```python
from build123d import *

# Parameters (mm, degrees)
SKETCH_1_R               = 21
EXTRUDE_1_DEPTH          = 25
CUT_EXTRUDE_1_DEPTH      = 396.281407624
CUT_EXTRUDE_1_DEPTH_BACK = 396.281407624
SKETCH_2_W               = 10
SKETCH_2_H               = 16.9


with BuildPart() as part:
    # 草图1 → 凸台-拉伸1 (new, symmetric)
    with BuildSketch(Plane.XY):
        with BuildLine():
            Line((0, 0), (0, 121.205505282))
            ThreePointArc((0, 121.205505282), (5, 143), (0, 164.794494718))
            Line((0, 164.794494718), (0, 370))
            Line((0, 370), (-15, 385))
            Line((-15, 385), (-90, 374.459437397))
            Line((-90, 374.459437397), (-90, 164.794494718))
            ThreePointArc((-90, 164.794494718), (-95, 143), (-90, 121.205505282))
            Line((-90, 121.205505282), (-90, 90))
            ThreePointArc((-90, 90), (-63.639610307, 26.360389693), (0, 0))
        make_face()
        with Locations((-45, 143)):
            Circle(SKETCH_1_R, mode=Mode.SUBTRACT)
    extrude(amount=EXTRUDE_1_DEPTH, both=True)

    # 草图2 → 切除-拉伸1 (cut, two sides: drawn at the far end of the back side and taken through both)
    with BuildSketch(Plane(origin=(-36.649271725, -5.150719239, 0), x_dir=(0, 0, -1), z_dir=(0.9902680687415697, 0.1391731009600695, 0)).offset(-CUT_EXTRUDE_1_DEPTH_BACK)):
        with Locations((-20, 374.89080298)):
            Rectangle(SKETCH_2_W, SKETCH_2_H)
        with Locations((20, 374.89080298)):
            Rectangle(SKETCH_2_W, SKETCH_2_H)
    extrude(amount=CUT_EXTRUDE_1_DEPTH + CUT_EXTRUDE_1_DEPTH_BACK, mode=Mode.SUBTRACT)


solid = part.part
```
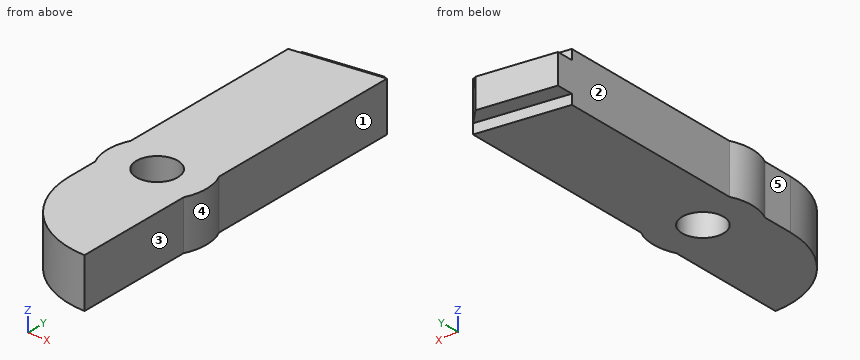
The listing builds one solid part. Answer for the finished solid, in the listing's coordinates (mm). Face numbers are marked on the shaded views. A direction names the side the tool comes from. Give positions to 0.01 mm unless a question says otherwise; leave off trailing zeros. Loops run counter-clockwise (first coordinate to the right, second up) from the corner with the lowest first, then second, coordinate; pieces in that order, holes last. Notation, with made-up numbers: (-34.75, 84) - (-0.75, 84) arc R34 ccw to (-0.75, 115) - close; hole circle Ø2 at (35, 46). An arc over 180 degrees is marked (long way). Answer as CSV lines item,"result". Start each with the question number.
Item 1: Each of these flat-tipped pins is pushed along its axis until it touches: pin 1 (2 mm diameter, centred on y = 176, z = 14, fed in from -X); pin 2 (6 mm diameter, centred on x = -55.5, z = 2.5, fed in from +Y); pin 3 (5 mm diameter, centred on x = -64.5, z = 19.5, fed in from -Y). Where does it stop, or does it pass through?
Item 2: A cutting plane is placed at C-C on x = -45. Determine the outline of the cut face in (y, z), then the cut area to 3 significant figures.
Item 3: Find the intervals of material crossed by line 1 (X direction, y = 318, z = 16); line 2 (X direction, y = 159, z = 22.5); line 3 (Y direction, x = -35, z = -13.5), in increasing order. Write a range as from..to.
Item 4: A cutting plane is placed at B-B on z = 6. Determine the outline of the cut face in (x, y).
Item 5: A cutting plane is placed at D-D on y = 274. Determine the outline of the cut face in (x, z), then the cut area to 3 significant figures.
Item 6: For the marked faces 1, 2, 3, 4 and 5, determine the directions among +Z, -Z, +X, -X, +Y, -Y from which every point of the face is accessible in a straight line to the end or side of a thin tool.
Item 7: A cutting plane is placed at A-A on y = 143. Determine the outline of the cut face in (x, z), then the cut area to 3 significant figures.
Found:
1,pin 1,"stops at x = -90"
1,pin 2,"stops at y = 379.73"
1,pin 3,"stops at y = 24.76"
2,outline,"(12.06, -25) - (122, -25) - (122, 25) - (12.06, 25) - close; (164, -25) - (363.72, -25) - (363.72, -15) - (380.78, -15) - (380.78, 15) - (363.72, 15) - (363.72, 25) - (164, 25) - close"
2,area,"16,000 mm^2"
3,line 1,"x = -90..0"
3,line 2,"x = -92.37..-58.6, -31.4..2.37"
3,line 3,"y = 7.08..124.53, 161.47..382.19"
4,outline,"(-90, 90) arc R90 ccw to (0, 0) - (0, 121.21) arc R50 ccw to (0, 164.79) - (0, 370) - (-15, 385) - (-90, 374.46) - (-90, 164.79) arc R50 ccw to (-90, 121.21) - close; hole circle Ø42 at (-45, 143)"
5,outline,"(-90, -25) - (0, -25) - (0, 25) - (-90, 25) - close"
5,area,"4,500 mm^2"
6,face 1,"+Z, -Z, +X, +Y"
6,face 2,"+Z, -Z, -X, +Y"
6,face 3,"+Z, -Z, +X, -Y"
6,face 4,"+Z, -Z, +X"
6,face 5,"+Z, -Z, -X, -Y"
7,outline,"(-95, -25) - (-66, -25) - (-66, 25) - (-95, 25) - close; (-24, -25) - (5, -25) - (5, 25) - (-24, 25) - close"
7,area,"2,900 mm^2"
